Design review of the part built by this model. Coordinates are the model's own, in mm. Face numbers are marked on the shaded views. Give positions to 0.01 mm unless a question says otherwise; leave off trailing zeros. Write each loop counter-clockwise with the first axis right and the second up, starting at its lowest first coordinate (ties: lowest second). Pieces come first, ordered by that corner, then holes. Notation, with made-up numbers: (-3, -25) -> (18, -25) arc R15 ccw to (18, -3) -> close; hole circle Ø10 at (30, -9). An arc over 180 degrees is marked (long way). Use CSV: the item, a comma, the result in double quotes.
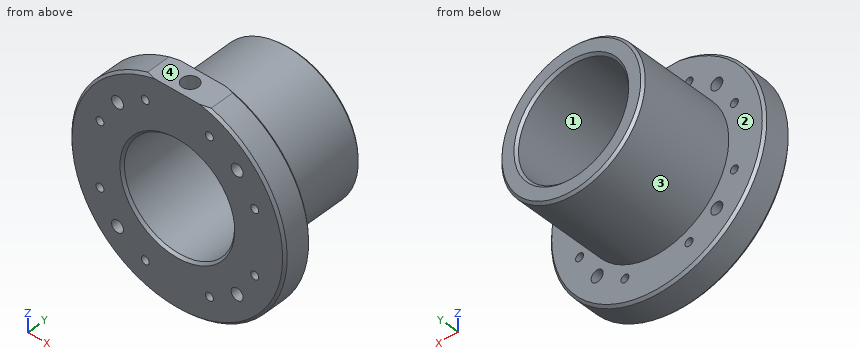
```python
from build123d import *

# Parameters (mm, degrees)
SKETCH1_R              = 45
BOSS_EXTRUDE1_DEPTH    = 12
SKETCH2_R              = 30
BOSS_EXTRUDE2_DEPTH    = 40
SKETCH3_R              = 23
CUT_EXTRUDE1_DEPTH     = 83.182723245
CHAMFER1_SIZE          = 1
M6_TAPPED_HOLE1_D      = 5
M4_TAPPED_HOLE1_D      = 3.3
CUT_EXTRUDE2_DEPTH     = 83.182723245
CIRPATTERN1_COUNT      = 8
M8_TAPPED_HOLE1_REACH  = 113.683
M8_TAPPED_HOLE1_BORE_R = 3.4


with BuildPart() as part:
    # Sketch1 → Boss-Extrude1 (new body)
    with BuildSketch(Plane(origin=(0, 0, 0), x_dir=(1, 0, 0), z_dir=(0, 1, 0))):
        with Locations(Location((0, 0, 0), (0, 0, 270))):
            Circle(SKETCH1_R)
    extrude(amount=BOSS_EXTRUDE1_DEPTH)

    # Sketch2 → Boss-Extrude2 (add)
    with BuildSketch(Plane(origin=(0, 12, 0), x_dir=(1, 0, 0), z_dir=(0, 1, 0))):
        with Locations(Location((0, 0, 0), (0, 0, 270))):
            Circle(SKETCH2_R)
    extrude(amount=BOSS_EXTRUDE2_DEPTH)

    # Sketch3 → Cut-Extrude1 (cut, through all)
    with BuildSketch(Plane.XZ):
        with Locations(Location((0, 0, 0), (0, 0, 270))):
            Circle(SKETCH3_R)
    extrude(amount=-CUT_EXTRUDE1_DEPTH, mode=Mode.SUBTRACT)

    # Chamfer1
    chamfer1_edges = [part.edges().sort_by_distance(p)[0] for p in [
        (0, 52, 23),
        (0, 0, 23),
        (0, 0, -45),
        (0, 12, -45),
        (0, 52, -30),
    ]]
    chamfer(chamfer1_edges, length=CHAMFER1_SIZE)

    # M6 Tapped Hole1 (through all)
    with Locations(Plane(origin=(0, 0, 0), x_dir=(-1, 0, 0), z_dir=(0, -1, 0))):
        with Locations((25, -25), (-25, -25), (-25, 25), (25, 25)):
            Hole(M6_TAPPED_HOLE1_D / 2)

    # M4 Tapped Hole1 (through all)
    with Locations(Plane(origin=(0, 0, 0), x_dir=(-1, 0, 0), z_dir=(0, -1, 0))):
        with Locations((13.393920133, -32.335783638)):
            m4_tapped_hole1 = Hole(M4_TAPPED_HOLE1_D / 2)

    # Sketch8 → Cut-Extrude2 (cut, through all)
    with BuildSketch(Plane.XZ):
        with BuildLine():
            Line((-13.266499161, 43), (13.266499161, 43))
            ThreePointArc((13.266499161, 43), (0, 45), (-13.266499161, 43))
        make_face()
    extrude(amount=-CUT_EXTRUDE2_DEPTH, mode=Mode.SUBTRACT)

    # CirPattern1: M4 Tapped Hole1 ×8 about axis
    cirpattern1_axis = Axis((0, 0, 0), (0, 1, 0))
    for i in range(1, CIRPATTERN1_COUNT):
        add(m4_tapped_hole1.rotate(cirpattern1_axis, i * 360 / CIRPATTERN1_COUNT), mode=Mode.SUBTRACT)

    # M8 Tapped Hole1 bore → M8 Tapped Hole1 (cut, up to next)
    with BuildSketch(Plane.XY.offset(43), mode=Mode.PRIVATE) as m8_tapped_hole1_sk1:
        with Locations((0, 6)):
            Circle(M8_TAPPED_HOLE1_BORE_R)
    m8_tapped_hole1_tool1 = extrude(m8_tapped_hole1_sk1.sketch, amount=-M8_TAPPED_HOLE1_REACH, mode=Mode.PRIVATE) & part.part
    add(m8_tapped_hole1_tool1.solids().sort_by_distance((0, 6, 43))[0], mode=Mode.SUBTRACT)


solid = part.part
```
(1) Mouldability with a two-part tool opening along Z and no side actions: class the marked faces 1, 2, 3 and 4 as +Z half, -Z half, draft (parallel to the pull), parting line (faces both ways), or undercut.
Established:
face 1,"undercut"
face 2,"draft"
face 3,"parting line"
face 4,"+Z half"
(2) For line 1 along Z through (x, y) = (1, 26.5); line 2 along Z through (x, y) = (-25, 2.75), list the stretches that pass through material, from the lowest coordinate up. Write a range as [from, to].
Established:
line 1,"z = [-29.98, -22.98], [22.98, 29.98]"
line 2,"z = [-37.42, -27.5], [-22.5, 22.5], [27.5, 37.42]"
(3) Take a section at C-C (y = 6). State how many separate pieces and enclosed holes the cut face has, then the cut area to 3 significant figures.
Established:
separate pieces,"1"
enclosed holes,"12"
area,"4,380 mm2"
(4) Take a section at D-D (y = 21.5). Write out the cut boundary in (x, z), then the cut area to 3 significant figures.
Established:
outline,"circle Ø60 at (0, 0); hole circle Ø46 at (0, 0)"
area,"1,170 mm2"
(5) Take a section at A-A (z = 0). Write out the cut boundary in (x, y).
Established:
outline,"(-45, 1) -> (-44, 0) -> (-24, 0) -> (-23, 1) -> (-23, 51) -> (-24, 52) -> (-29, 52) -> (-30, 51) -> (-30, 12) -> (-44, 12) -> (-45, 11) -> close; (23, 1) -> (24, 0) -> (44, 0) -> (45, 1) -> (45, 11) -> (44, 12) -> (30, 12) -> (30, 51) -> (29, 52) -> (24, 52) -> (23, 51) -> close"
(6) Clearance check with flat-ended pins moving along their axes: pin 1 (3 mm diameter, centred on x = 13.39, z = -32.34, fed in from +Y); pin 2 (1 mm diameter, centred on x = 11.5, y = 34.5, fed in from -Z); pin 3 (5.5 mm diameter, centred on x = 32.34, z = 13.39, fed in from +Y); pin 4 (3 mm diameter, centred on y = 19.5, z = -1, fed in from -X). State where each tip first meets the part, or that it passes through.
Established:
pin 1,"passes through"
pin 2,"stops at z = -27.91"
pin 3,"stops at y = 12"
pin 4,"stops at x = -30"
(7) Take a section at B-B (x = 0). Write out the cut boundary in (y, z).
Established:
outline,"(0, -44) -> (1, -45) -> (11, -45) -> (12, -44) -> (12, -30) -> (51, -30) -> (52, -29) -> (52, -24) -> (51, -23) -> (1, -23) -> (0, -24) -> close; (0, 24) -> (1, 23) -> (2.6, 23) -> (2.6, 43) -> (0, 43) -> close; (9.4, 23) -> (51, 23) -> (52, 24) -> (52, 29) -> (51, 30) -> (12, 30) -> (12, 43) -> (9.4, 43) -> close"
